Can you work these out from the model? Positions are in its coordinate system, mm. A direction names the side the tool comes from. Round coordinates to 2 decimals unless told otherwise and drop trailing zeros. Write each loop counter-clockwise with the first axis right and the second up, starting at its lowest first coordinate (ties: lowest second). Pieces come first, ordered by that corner, then holes. Notation, with made-up numbers: (81.25, -37.75) -> (129.25, -37.75) arc R8 ccw to (129.25, -27.75) -> close; hole circle Ø2 at (-10.75, 23). An arc over 180 degrees is marked (long way). Write item = value, one per line. Start each with the question number.
1) Imagine slicing it at C-C, the plane x = 6. State how many separate pieces and enclosed holes the cut face has, then the cut area to 3 significant figures.
2) If I drill on line 1 (Z direction, x = 6, y = 4.5); line 2 (Z direction, x = 6, y = 7.7); line 3 (X direction, y = 4, z = -90), over which ranges is the centre line in solid material (lowest first)?
3) Thinking about a two-plate mould opening in Y: for faces 1 (the face through (6.1, 70.1, -12.3)), 2 (the face through (6, 0, -51)), 3 (the face through (7.08, 75.12, -9.19)), which applies, +Y half, -Y half, draft (parallel to the pull), parting line (faces both ways), or undercut?
4) For faces 4 (the face through (3.8, 77.8, -6.3)), 5 (the face through (6, 96, -12)), 6 (the face through (8.2, 6.3, -67.8)), which set-ups out of +Z, -Z, +X, -X, +Y, -Y let a thin tool reach every point of the face, with its end or its side?
5) Imagine slicing it at A-A, the plane y = 80. Please give me the cut outline in (x, z), then the cut area to 4 significant figures.
6) Imagine slicing it at D-D, the plane y = 24. Please give me the cut outline in (x, z), then the cut area to 3 significant figures.
7) Imagine slicing it at B-B, the plane z = -70. Please give me the cut outline in (x, y), then the cut area to 4 significant figures.
8) I'm going to push flat-ended pins straight in: pin 1 (3.5 mm diameter, centred on x = 9, z = -74, fed in from +Y); pin 2 (6 mm diameter, centred on x = 6, y = 110, fed in from -Z); pin 3 (4 mm diameter, centred on x = 10, y = 76.5, fed in from -Z). Where does each tip first touch, or does it pass through?
from build123d import *

# Parameters (mm, degrees)
BOSS_EXTRUDE1_DEPTH                                  = 12
CUT_EXTRUDE1_DEPTH                                   = 157.665248221
CBORE_FOR_M5_HEXAGON_SOCKET_HEAD_CAP_SCR_D           = 5.5
CBORE_FOR_M5_HEXAGON_SOCKET_HEAD_CAP_SCR_CBORE_D     = 10
CBORE_FOR_M5_HEXAGON_SOCKET_HEAD_CAP_SCR_CBORE_DEPTH = 5.7
CBORE_FOR_M5_HEXAGON_SOCKET_HEAD_CAP_2_D             = 5.5
CBORE_FOR_M5_HEXAGON_SOCKET_HEAD_CAP_2_CBORE_D       = 10
CBORE_FOR_M5_HEXAGON_SOCKET_HEAD_CAP_2_CBORE_DEPTH   = 5.7
CHAMFER1_SIZE                                        = 1
FILLET1_R                                            = 5


with BuildPart() as part:
    # Sketch1 → Boss-Extrude1 (new body)
    with BuildSketch(Plane(origin=(0, 0, 0), x_dir=(0, 0, -1), z_dir=(1, 0, 0))):
        Polygon((0, 0), (0, 120), (12, 120), (12, 70), (60, 12), (100, 12), (100, 0), align=None)
    extrude(amount=BOSS_EXTRUDE1_DEPTH)

    # Sketch2 → Cut-Extrude1 (cut, through all)
    with BuildSketch(Plane(origin=(12, 0, 0), x_dir=(0, 0, -1), z_dir=(1, 0, 0))):
        with BuildLine():
            Line((12, 37.294498848), (12, 17))
            ThreePointArc((12, 17), (13.464466094, 13.464466094), (17, 12))
            Line((17, 12), (33.795447323, 12))
            ThreePointArc((33.795447323, 12), (38.319781133, 14.871525529), (37.647418928, 20.18783857))
            Line((37.647418928, 20.18783857), (20.851971606, 40.482337418))
            ThreePointArc((20.851971606, 40.482337418), (15.305871615, 41.998744698), (12, 37.294498848))
        make_face()
    extrude(amount=-CUT_EXTRUDE1_DEPTH, mode=Mode.SUBTRACT)

    # CBORE for M5 Hexagon socket head cap scr (through all)
    with Locations(Plane(origin=(0, 0, -12), x_dir=(-1, 0, 0), z_dir=(0, 0, -1))):
        with Locations((-6, 80), (-6, 110)):
            CounterBoreHole(CBORE_FOR_M5_HEXAGON_SOCKET_HEAD_CAP_SCR_D / 2, CBORE_FOR_M5_HEXAGON_SOCKET_HEAD_CAP_SCR_CBORE_D / 2, CBORE_FOR_M5_HEXAGON_SOCKET_HEAD_CAP_SCR_CBORE_DEPTH)

    # CBORE for M5 Hexagon socket head cap 2 (through all)
    with Locations(Plane(origin=(0, 12, 0), x_dir=(1, 0, 0), z_dir=(0, 1, 0))):
        with Locations((6, 70), (6, 90)):
            CounterBoreHole(CBORE_FOR_M5_HEXAGON_SOCKET_HEAD_CAP_2_D / 2, CBORE_FOR_M5_HEXAGON_SOCKET_HEAD_CAP_2_CBORE_D / 2, CBORE_FOR_M5_HEXAGON_SOCKET_HEAD_CAP_2_CBORE_DEPTH)

    # Chamfer1
    chamfer1_edges = [part.edges().sort_by_distance(p)[0] for p in [
        (12, 120, -6),
        (0, 120, -6),
        (12, 6, -100),
        (0, 6, -100),
    ]]
    chamfer(chamfer1_edges, length=CHAMFER1_SIZE)

    # Fillet1
    fillet1_edges = [part.edges().sort_by_distance(p)[0] for p in [
        (6, 70, -12),
        (6, 12, -60),
    ]]
    fillet(fillet1_edges, radius=FILLET1_R)


solid = part.part
Reported:
q1.separate_pieces = 5
q1.enclosed_holes = 1
q1.area = 2,960 mm²
q2.line_1 = -100 to -92.75, -87.25 to -72.75, -67.25 to 0
q2.line_2 = -100 to -95, -85 to -75, -65 to 0
q2.line_3 = 0 to 3.25, 8.75 to 12
q3.face_1 = +Y half
q3.face_2 = -Y half
q3.face_3 = undercut
q4.face_4 = -Z
q4.face_5 = -Z, +X, -X, +Y
q4.face_6 = +Y
q5.outline = (0, -12) -> (1, -12) -> (1, -6.3) -> (3.25, -6.3) -> (3.25, 0) -> (0, 0) -> close; (8.75, -6.3) -> (11, -6.3) -> (11, -12) -> (12, -12) -> (12, 0) -> (8.75, 0) -> close
q5.area = 52.35 mm²
q6.outline = (0, -50.07) -> (12, -50.07) -> (12, -34.49) -> (0, -34.49) -> close; (0, -12) -> (12, -12) -> (12, 0) -> (0, 0) -> close
q6.area = 331 mm²
q7.outline = (0, 0) -> (3.25, 0) -> (3.25, 6.3) -> (1, 6.3) -> (1, 12) -> (0, 12) -> close; (8.75, 0) -> (12, 0) -> (12, 12) -> (11, 12) -> (11, 6.3) -> (8.75, 6.3) -> close
q7.area = 52.35 mm²
q8.pin_1 = 12
q8.pin_2 = -6.3
q8.pin_3 = -12
